from build123d import *

# Parameters (mm, degrees)
BOSS_EXTRUDE1_DEPTH          = 400
SKETCH2_W                    = 100
SKETCH2_H                    = 100
BOSS_EXTRUDE2_DEPTH          = 5
F_10_5_10_5_DIAMETER_HOLE1_D = 10.5
BOSS_EXTRUDE3_DEPTH          = 200
SKETCH6_W                    = 100
SKETCH6_H                    = 100
BOSS_EXTRUDE4_DEPTH          = 5
BOSS_EXTRUDE5_DEPTH          = 195
CUT_EXTRUDE1_DEPTH           = 20
CUT_EXTRUDE1_DEPTH_BACK      = 20
F_18_5_18_5_DIAMETER_HOLE1_D = 18.5


with BuildPart() as part:
    # Sketch1 → Boss-Extrude1 (new body)
    with BuildSketch(Plane.XY):
        with BuildLine():
            Line((0, 0), (0, 49))
            ThreePointArc((0, 49), (0.292893219, 49.707106781), (1, 50))
            Line((1, 50), (99, 50))
            ThreePointArc((99, 50), (99.707106781, 49.707106781), (100, 49))
            Line((100, 49), (100, 0))
            Line((100, 0), (95, 0))
            Line((95, 0), (92.790644836, 42.157007869))
            ThreePointArc((92.790644836, 42.157007869), (91.859819959, 44.176123113), (89.794756232, 45))
            Line((89.794756232, 45), (10.205243768, 45))
            ThreePointArc((10.205243768, 45), (8.140180041, 44.176123113), (7.209355164, 42.157007869))
            Line((7.209355164, 42.157007869), (5, 0))
            Line((5, 0), (0, 0))
        make_face()
    extrude(amount=BOSS_EXTRUDE1_DEPTH)

    # Sketch2 → Boss-Extrude2 (add)
    with BuildSketch(Plane.XZ):
        with Locations((50, 400)):
            Rectangle(SKETCH2_W, SKETCH2_H)
        with Locations((50, 0)):
            Rectangle(SKETCH2_W, SKETCH2_H)
    extrude(amount=BOSS_EXTRUDE2_DEPTH)

    # Ø10.5 (10.5) Diameter Hole1 (through all)
    with Locations(Plane(origin=(0, 0, 0), x_dir=(1, 0, 0), z_dir=(0, 1, 0))):
        with Locations((17.5, -425), (82.5, -425), (83.148664141, 25), (17.5, 25)):
            Hole(F_10_5_10_5_DIAMETER_HOLE1_D / 2)

    # Sketch5 → Boss-Extrude3 (add)
    with BuildSketch(Plane(origin=(0, 50, 0), x_dir=(1, 0, 0), z_dir=(0, 1, 0))):
        with BuildLine():
            Line((1, -350), (99, -350))
            ThreePointArc((99, -350), (99.707106781, -350.292893219), (100, -351))
            Line((100, -351), (100, -400))
            Line((100, -400), (95, -400))
            Line((95, -400), (92.6913149, -355.947664044))
            ThreePointArc((92.6913149, -355.947664044), (92.381039941, -355.274625629), (91.692685366, -355))
            Line((91.692685366, -355), (8.307314634, -355))
            ThreePointArc((8.307314634, -355), (7.618960059, -355.274625629), (7.3086851, -355.947664044))
            Line((7.3086851, -355.947664044), (5, -400))
            Line((5, -400), (0, -400))
            Line((0, -400), (0, -351))
            ThreePointArc((0, -351), (0.292893219, -350.292893219), (1, -350))
        make_face()
    extrude(amount=BOSS_EXTRUDE3_DEPTH)

    # Sketch6 → Boss-Extrude4 (add)
    with BuildSketch(Plane(origin=(0, 50, 0), x_dir=(1, 0, 0), z_dir=(0, 1, 0))):
        with Locations((50, -50)):
            Rectangle(SKETCH6_W, SKETCH6_H)
    extrude(amount=BOSS_EXTRUDE4_DEPTH)

    # Sketch7 → Boss-Extrude5 (add)
    with BuildSketch(Plane(origin=(0, 55, 0), x_dir=(1, 0, 0), z_dir=(0, 1, 0))):
        with BuildLine():
            Line((1, -50), (99, -50))
            ThreePointArc((99, -50), (99.707106781, -50.292893219), (100, -51))
            Line((100, -51), (100, -100))
            Line((100, -100), (95, -100))
            Line((95, -100), (92.6913149, -55.947664044))
            ThreePointArc((92.6913149, -55.947664044), (92.381039941, -55.274625629), (91.692685366, -55))
            Line((91.692685366, -55), (8.307314634, -55))
            ThreePointArc((8.307314634, -55), (7.618960059, -55.274625629), (7.3086851, -55.947664044))
            Line((7.3086851, -55.947664044), (5, -100))
            Line((5, -100), (0, -100))
            Line((0, -100), (0, -51))
            ThreePointArc((0, -51), (0.292893219, -50.292893219), (1, -50))
        make_face()
    extrude(amount=BOSS_EXTRUDE5_DEPTH)

    # Sketch8 → Cut-Extrude1 (cut, two sides: drawn at the far end of the back side and taken through both)
    with BuildSketch(Plane(origin=(0, 50, 0), x_dir=(1, 0, 0), z_dir=(0, 1, 0)).offset(-CUT_EXTRUDE1_DEPTH_BACK)):
        with BuildLine():
            Line((20.75, -37.5), (20.75, -12.5))
            ThreePointArc((20.75, -12.5), (25, -8.25), (29.25, -12.5))
            Line((29.25, -12.5), (29.25, -37.5))
            ThreePointArc((29.25, -37.5), (25, -41.75), (20.75, -37.5))
        make_face()
        with BuildLine():
            Line((70.75, -37.5), (70.75, -12.5))
            ThreePointArc((70.75, -12.5), (75, -8.25), (79.25, -12.5))
            Line((79.25, -12.5), (79.25, -37.5))
            ThreePointArc((79.25, -37.5), (75, -41.75), (70.75, -37.5))
        make_face()
    extrude(amount=CUT_EXTRUDE1_DEPTH + CUT_EXTRUDE1_DEPTH_BACK, mode=Mode.SUBTRACT)

    # Ø18.5 (18.5) Diameter Hole1 (through all)
    with Locations(Plane(origin=(0, 0, 50), x_dir=(-1, 0, 0), z_dir=(0, 0, -1))):
        with Locations((-50, 220)):
            Hole(F_18_5_18_5_DIAMETER_HOLE1_D / 2)


solid = part.part
The listing builds one solid part. Answer for the finished solid, in the listing's coordinates (mm). A direction names the side the tool comes from. Give positions to 0.01 mm unless a question says otherwise; leave off trailing zeros. Order: outer loops, then holes, each group sorted by start corner. A loop starts at its lowest first (then second) coordinate and runs counter-clockwise, first axis right, second up. Notation, with made-up numbers: (-8.75, 61) - (22.25, 61) arc R20 ccw to (22.25, 85) - close; hole circle Ø8 at (19, -29). An arc over 180 degrees is marked (long way). One line per item, written item: value. Start each with the question number.
1) A tool of negligible diameter and unlimited length cuts with its end or side. For faces 5 (the face through (70.75, 50, 25)), 6 (the face through (49, 55, 25)), 7 (the face through (49, -5, 1)), 8 (the face through (98, 120, 100)), 9 (the face through (43.18, 226.25, 52.53)), from which of +Z, -Z, +X, -X, +Y, -Y can it reach the whole face along a straight path? Write none if from no direction.
2) The mould has two halves that part along Z. Classify faces 1 (the face through (21.67, -2.53, -21.81)), 2 (the face through (6.12, 21.37, 197.2)), 3 (the face through (49, 151, 50)), 4 (the face through (6.17, 148.6, 377.67)): released by +Z, released by -Z, zero draft, split by the parting line, or undercut.
3) Given pin 1 Ø4 at (x, z) = (98.5, 246) entering from -Y; pin 2 Ø4 at (x, z) = (89, 291) entering from +Y; pin 3 Ø21.5 at (x, y) = (50, 220) entering from +Z, each flat-ended and moving along its own axis, determine where each tip first touches the part or whether it passes through.
4) Find the intervals of material crossed by L1, parallel to X at y = -1, z = 425; L2, parallel to Z at x = 42.5, y = 138.5; L3, parallel to X at y = 227, z = 359, in increasing order.
5) A cutting plane is placed at A-A on x = 50. State how many separate pieces and enclosed holes the cut face has, then the cut area to 3 significant figures.
6) A cutting plane is placed at B-B on y = 105. Give the vertices of the cut face in (x, z).
7) A cutting plane is placed at C-C on z = -25. Give the vertices of the cut face in (x, y).
Answer sheet:
1. face 5: +Y
1. face 6: -Z, +X, -X, +Y
1. face 7: +Z, -Z, +X, -X, -Y
1. face 8: +X, -X, +Y
1. face 9: +Z, -Z
2. face 1: undercut
2. face 2: zero draft
2. face 3: released by -Z
2. face 4: released by +Z
3. pin 1: stops at y = 0
3. pin 2: stops at y = 50
3. pin 3: stops at z = 355
4. L1: x = 0 to 12.25, 22.75 to 77.25, 87.75 to 100
4. L2: z = 50 to 55, 350 to 355
4. L3: x = 0 to 7.15, 92.85 to 100
5. separate pieces: 5
5. enclosed holes: 0
5. area: 5,290 mm2
6. outline: (0, 51) arc R1 ccw to (1, 50) - (99, 50) arc R1 ccw to (100, 51) - (100, 100) - (95, 100) - (92.69, 55.95) arc R1 cw to (91.69, 55) - (8.31, 55) arc R1 cw to (7.31, 55.95) - (5, 100) - (0, 100) - close; (0, 351) arc R1 ccw to (1, 350) - (99, 350) arc R1 ccw to (100, 351) - (100, 400) - (95, 400) - (92.69, 355.95) arc R1 cw to (91.69, 355) - (8.31, 355) arc R1 cw to (7.31, 355.95) - (5, 400) - (0, 400) - close
7. outline: (0, -5) - (12.25, -5) - (12.25, 0) - (0, 0) - close; (22.75, -5) - (77.9, -5) - (77.9, 0) - (22.75, 0) - close; (88.4, -5) - (100, -5) - (100, 0) - (88.4, 0) - close
